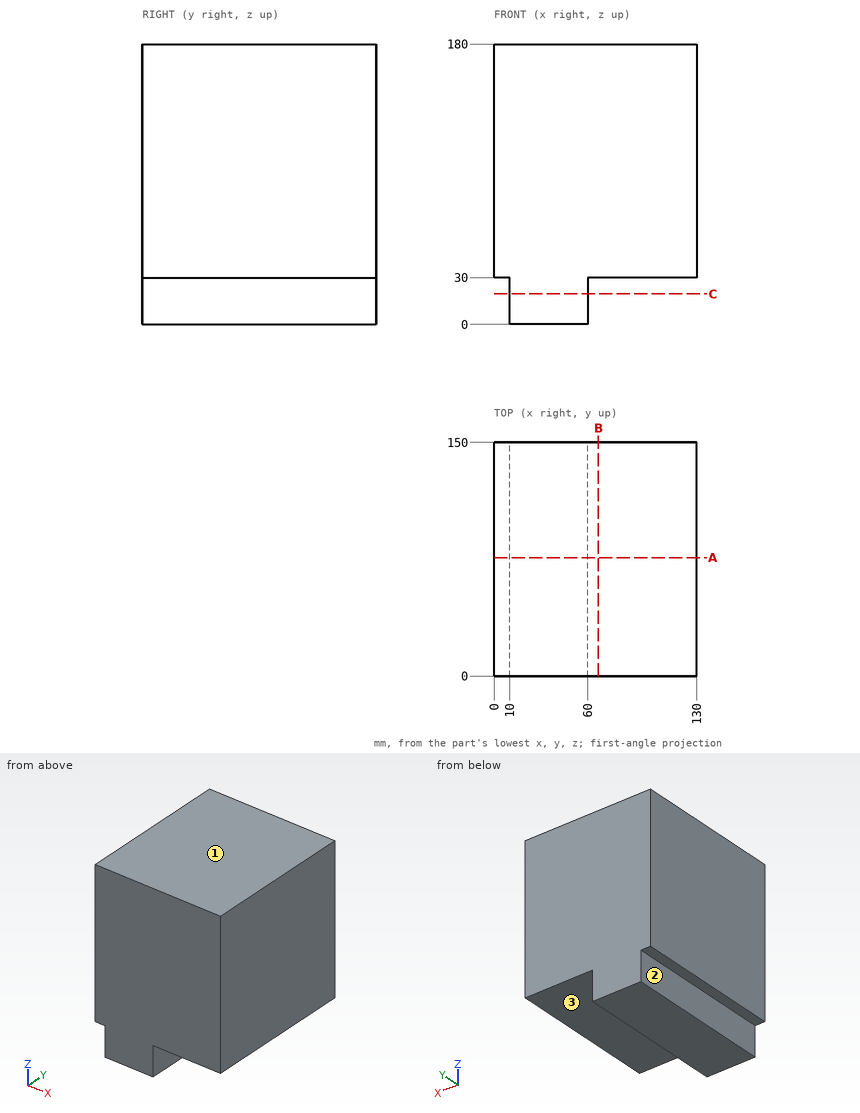
Job drawing, mm, ordinate dimensions from the low corner. One solid piece. A direction names the side the tool comes from. Round coordinates to 2 decimals unless told otherwise and drop trailing zeros. Loops run counter-clockwise (first coordinate to the right, second up) from the corner with the lowest first, then second, coordinate; pieces in that order, holes last. Notation, with made-up numbers: (43, 42.5) -> (94, 42.5) arc R24 cw to (94, 73.5) -> close; hole circle Ø9 at (54, 77.25). An arc over 180 degrees is marked (long way). Use a Markdown table: item, result.
1) Cut at C-C, the plane z = 19.5. List the corners of the cut face in (x, y), and give its area (3 significant figures).
The answers:
| item | result |
|---|---|
| outline | (10, 0) -> (60, 0) -> (60, 150) -> (10, 150) -> close |
| area | 7,500 mm2 |
2) Probe line 1 (Z direction, x = 6.5, y = 136); line 2 (X direction, y = 16, z = 10). List the from-to ranges inside material, lowest first. Write a range as [from, to].
The answers:
| item | result |
|---|---|
| line 1 | z = [30, 180] |
| line 2 | x = [10, 60] |
3) Cut at B-B, the plane x = 67. List the corners of the cut face in (y, z).
The answers:
| item | result |
|---|---|
| outline | (0, 30) -> (150, 30) -> (150, 180) -> (0, 180) -> close |
4) Drop flat-ended pins along their axis: pin 1 Ø9 at (y, z) = (42.5, 11.5) entering from +X; pin 2 Ø5 at (x, y) = (3, 98.5) entering from -Z. Give the stop position or say it passes through.
The answers:
| item | result |
|---|---|
| pin 1 | stops at x = 60 |
| pin 2 | stops at z = 30 |
5) Cut at A-A, the plane y = 76. List the corners of the cut face in (x, z).
The answers:
| item | result |
|---|---|
| outline | (0, 30) -> (10, 30) -> (10, 0) -> (60, 0) -> (60, 30) -> (130, 30) -> (130, 180) -> (0, 180) -> close |
6) Tool access for the marked faces 1, 2 and 3: list every direction of +Z, -Z, +X, -X, +Y, -Y with a clear straight run to the whole face (end or side of a thin tool).
The answers:
| item | result |
|---|---|
| face 1 | +Z, +X, -X, +Y, -Y |
| face 2 | -Z, -X, +Y, -Y |
| face 3 | -Z, +X, +Y, -Y |
